Check sheet for the modelled part. Datum: model origin and axes. Units: mm. Face numbers are marked on the shaded views. A direction names the side the tool comes from. Round coordinates to 2 decimals unless told otherwise and drop trailing zeros. Order: outer loops, then holes, each group sorted by start corner. A loop starts at its lowest first (then second) coordinate and runs counter-clockwise, first axis right, second up. Notation, with made-up numbers: (74.25, 35) -> (78.25, 35) arc R19 cw to (78.25, 65) -> close; hole circle Ø6 at (15.5, 81.25). An arc over 180 degrees is marked (long way). Answer in a Markdown table with one row per item. Add a question column.
1. Depth check by flat-ended pin: P1, Ø10, axis at x = -11, y = 139, coming from the +Z side; P2, Ø16.5, axis at x = 16, y = 103, coming from the +Z side; P3, Ø3, axis at x = -129, y = 195, coming from the +Z side. Enter the tip coordinate at first touch or a pass-through.
2. Draft check along Y on the marked faces 1, 2 and 3. Enter one of: +Y half, -Y half, draft (parallel to the pull), parting line (faces both ways), or undercut.
3. Access from +Z, -Z, +X, -X, +Y, -Y to the whole of each face (thin tool, end or side, straight path). Record for the marked faces 4, 5, 6 and 7.
4. Sectioned sample at D-D, the plane x = 198. Record the boundary of the cut face in (y, z), then the cut area to 3 significant figures.
5. Sectioned sample at A-A, the plane y = 13. Record the boundary of the cut face in (x, z), then the cut area to 3 significant figures.
6. Sectioned sample at B-B, the plane x = 25. Record the boundary of the cut face in (y, z), then the cut area to 3 significant figures.
7. Sectioned sample at C-C, the plane z = 120. Record the boundary of the cut face in (x, y).
8. Material ranges on L1, parallel to Y at x = -184.5, z = 25; L2, parallel to Y at x = -130.5, z = -79; L3, parallel to Y at x = -72, z = 133, recorded low to high. Write a range as from..to.
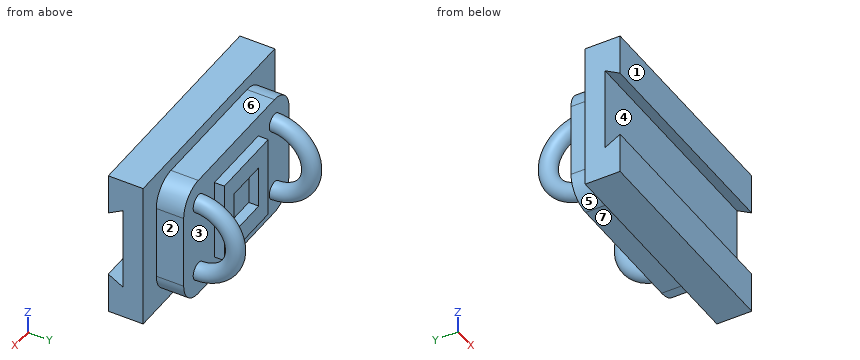
```python
from build123d import *

# Parameters (mm, degrees)
BASE_BLOCK_V_GROOVE_DEPTH   = 225
TOP_PAD_360X250_DEPTH       = 55
SQUARE_FRAME_SKETCH_150_W   = 150
SQUARE_FRAME_SKETCH_150_H   = 165
SQUARE_FRAME_SKETCH_150_W_2 = 85
SQUARE_FRAME_SKETCH_150_H_2 = 85
SQUARE_FRAME_BOSS_150_DEPTH = 20
LIFTING_HANDLE_35_PROFILE_R = 17.5


with BuildPart() as part:
    # Base V-Groove Profile Sketch → Base Block V-Groove (new, symmetric)
    with BuildSketch(Plane(origin=(0, 0, 0), x_dir=(0, 0, -1), z_dir=(1, 0, 0))):
        Polygon((-67.679491924, 0), (-85, 30), (85, 30), (67.679491924, 0), (150, 0), (150, 70), (-150, 70), (-150, 0), align=None)
    extrude(amount=BASE_BLOCK_V_GROOVE_DEPTH, both=True)

    # Top Pad Sketch 360x250 → Top Pad 360x250 (add)
    with BuildSketch(Plane(origin=(0, 70, 0), x_dir=(1, 0, 0), z_dir=(0, 1, 0))):
        with BuildLine():
            Line((-130, -125), (130, -125))
            ThreePointArc((130, -125), (165.355339059, -110.355339059), (180, -75))
            Line((180, -75), (180, 75))
            ThreePointArc((180, 75), (165.355339059, 110.355339059), (130, 125))
            Line((130, 125), (-130, 125))
            ThreePointArc((-130, 125), (-165.355339059, 110.355339059), (-180, 75))
            Line((-180, 75), (-180, -75))
            ThreePointArc((-180, -75), (-165.355339059, -110.355339059), (-130, -125))
        make_face()
    extrude(amount=TOP_PAD_360X250_DEPTH)

    # Square Frame Sketch 150 → Square Frame Boss 150 (add)
    with BuildSketch(Plane(origin=(0, 125, 0), x_dir=(1, 0, 0), z_dir=(0, 1, 0))):
        Rectangle(SQUARE_FRAME_SKETCH_150_W, SQUARE_FRAME_SKETCH_150_H)
        Rectangle(SQUARE_FRAME_SKETCH_150_W_2, SQUARE_FRAME_SKETCH_150_H_2, mode=Mode.SUBTRACT)
    extrude(amount=SQUARE_FRAME_BOSS_150_DEPTH)

    # Lifting Handle Ø35: sweep along a path in Handle Path Sketch
    with BuildLine(Plane(origin=(130, 0, 0), x_dir=(0, 0, -1), z_dir=(1, 0, 0))) as lifting_handle_35_path:
        ThreePointArc((-75, 125), (0, 200), (75, 125))
    # Lifting Handle Ø35 profile (on start of the path) → Lifting Handle Ø35 (sweep)
    with BuildSketch(Plane(origin=(130, 125, 75), x_dir=(0, 0, 1), z_dir=(0, 1, 0))):
        Circle(LIFTING_HANDLE_35_PROFILE_R)
    lifting_handle_35 = sweep(path=lifting_handle_35_path.line)

    # Lifting Handle Mirror: Lifting Handle Ø35 across plane
    add(lifting_handle_35.mirror(Plane(origin=(0, 0, 0), x_dir=(0, 0, 1), z_dir=(1, 0, 0))))


solid = part.part
```
Answer key:
| question | item | result |
|---|---|---|
| 1 | P1 | stops at z = 82.5 |
| 1 | P2 | stops at z = 125 |
| 1 | P3 | stops at z = 62.12 |
| 2 | face 1 | -Y half |
| 2 | face 2 | draft |
| 2 | face 3 | undercut |
| 3 | face 4 | +X, -X |
| 3 | face 5 | -Z, -X, +Y |
| 3 | face 6 | +Z, +X, -X, +Y |
| 3 | face 7 | -Z, +X, -X, +Y |
| 4 | outline | (0, -150) -> (70, -150) -> (70, 150) -> (0, 150) -> (0, 67.68) -> (30, 85) -> (30, -85) -> (0, -67.68) -> close |
| 4 | area | 16,400 mm² |
| 5 | outline | (-225, -150) -> (225, -150) -> (225, -75.19) -> (-225, -75.19) -> close; (-225, 75.19) -> (225, 75.19) -> (225, 150) -> (-225, 150) -> close |
| 5 | area | 67,300 mm² |
| 6 | outline | (0, -150) -> (70, -150) -> (70, -125) -> (125, -125) -> (125, -82.5) -> (145, -82.5) -> (145, -42.5) -> (125, -42.5) -> (125, 42.5) -> (145, 42.5) -> (145, 82.5) -> (125, 82.5) -> (125, 125) -> (70, 125) -> (70, 150) -> (0, 150) -> (0, 67.68) -> (30, 85) -> (30, -85) -> (0, -67.68) -> close |
| 6 | area | 31,800 mm² |
| 7 | outline | (-225, 0) -> (225, 0) -> (225, 70) -> (151.79, 70) -> (151.79, 125) -> (-151.79, 125) -> (-151.79, 70) -> (-225, 70) -> close |
| 8 | L1 | y = 30..70 |
| 8 | L2 | y = 0..19.61, 30..173.1 |
| 8 | L3 | y = 0..70 |
